Design review of the part built by this model. Coordinates are the model's own, in mm. Face numbers are marked on the shaded views. Round coordinates to 2 decimals unless told otherwise and drop trailing zeros. Loops run counter-clockwise (first coordinate to the right, second up) from the corner with the lowest first, then second, coordinate; pieces in that order, holes last. Notation, with made-up numbers: (52, 16) - (57, 16) arc R29 ccw to (57, 53) - close; hole circle Ø7 at (-29.5, 47). An arc over 180 degrees is marked (long way). Answer as CSV lines item,"result". Start each with the question number.
(1) Consider section C-C (x = 13.5). Give the boundary of the cut face in (y, z).
(2) Consider section A-A (y = 0). Give the boundary of the cut face in (x, z).
(3) Wall thickness on L1, parallel to Y at x = 50, z = 56.4; L2, parallel to Z at x = 0, y = 2.5: over which ranges is each line inside the solid? List them lowest first.
(4) Consider section B-B (z = -28). Give the boundary of the cut face in (x, y), and give its area (3 significant figures).
(5) Mouldability with a two-part tool opening along Z and no side actions: class the marked faces 1 and 2 as released by +Z, released by -Z, zero draft, split by the parting line, or undercut.
(6) For P1, Ø8, axis at y = -7.5, z = -10, coming from the +X side; P2, Ø1.5, axis at y = 1.5, z = 43.5, coming from the +X side; P3, Ø3, axis at x = 50, y = 5.5, coming from the -Z side, all flat-tipped, find the tip position at first contact; note any pin that passes through.
(7) Consider section D-D (x = 50). Give the boundary of the cut face in (y, z), and give its area (3 significant figures).
from build123d import *

# Parameters (mm, degrees)
EXTRUDE_1_DEPTH     = 12.5
SKETCH_3_R          = 2
CUT_EXTRUDE_1_DEPTH = 2


with BuildPart() as part:
    # 草图1 → 拉伸-薄壁1 (new, symmetric)
    with BuildSketch(Plane(origin=(0, 0, 0), x_dir=(1, 0, 0), z_dir=(0, 1, 0))):
        with BuildLine():
            ThreePointArc((23.666622657, -50.753236074), (-12.120618381, 54.672576399), (0, -56))
            Line((0, -56), (60, -56))
            Line((60, -56), (60, -58))
            Line((60, -58), (0, -58))
            ThreePointArc((0, -58), (-12.553497608, 56.625168413), (24.511859181, -52.565851648))
            Line((24.511859181, -52.565851648), (23.666622657, -50.753236074))
        make_face()
    extrude(amount=EXTRUDE_1_DEPTH, both=True)

    # 草图3 → 切除-拉伸1 (cut)
    with BuildSketch(Plane.XY.offset(58)):
        with Locations((50, 5.5)):
            Circle(SKETCH_3_R)
        with Locations(Location((50, -5.5, 0), (0, 0, 180))):
            Circle(SKETCH_3_R)
        with BuildLine():
            Line((15.5, 5.5), (29.5, 5.5))
            ThreePointArc((29.5, 5.5), (35, 0), (29.5, -5.5))
            Line((29.5, -5.5), (15.5, -5.5))
            ThreePointArc((15.5, -5.5), (10, 0), (15.5, 5.5))
        make_face()
    extrude(amount=-CUT_EXTRUDE_1_DEPTH, mode=Mode.SUBTRACT)


solid = part.part
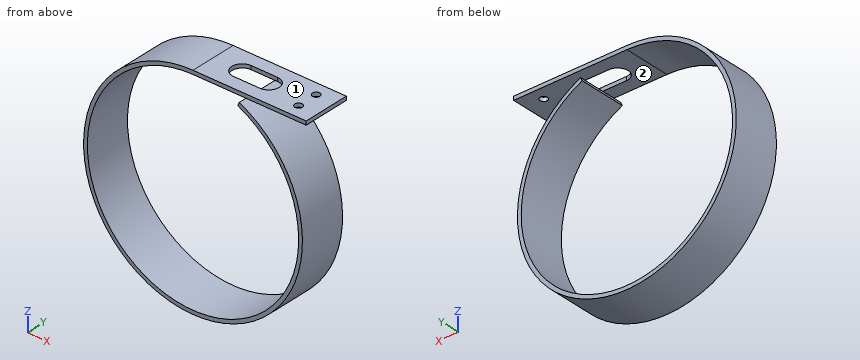
Determined:
1,outline,"(-12.5, -56.41) - (12.5, -56.41) - (12.5, -54.35) - (-12.5, -54.35) - close; (-12.5, 56) - (-5.12, 56) - (-5.12, 58) - (-12.5, 58) - close; (5.12, 56) - (12.5, 56) - (12.5, 58) - (5.12, 58) - close"
2,outline,"(0, 56) - (10, 56) - (10, 58) - (0, 58) arc R58 ccw (long way) to (24.51, 52.57) - (23.67, 50.75) arc R56 cw (long way) to start; (35, 56) - (60, 56) - (60, 58) - (35, 58) - close"
3,L1,"y = -12.5 to -7.5, -3.5 to 3.5, 7.5 to 12.5"
3,L2,"z = -58 to -56, 56 to 58"
4,outline,"(-50.79, -12.5) - (-48.5, -12.5) - (-48.5, 12.5) - (-50.79, 12.5) - close; (48.5, -12.5) - (50.79, -12.5) - (50.79, 12.5) - (48.5, 12.5) - close"
4,area,"115 mm^2"
5,face 1,"released by +Z"
5,face 2,"undercut"
6,P1,"stops at x = 57.69"
6,P2,"stops at x = 39.2"
6,P3,"stops at z = -31.81"
7,outline,"(-12.5, -29.39) - (12.5, -29.39) - (12.5, -25.22) - (-12.5, -25.22) - close; (-12.5, 25.22) - (12.5, 25.22) - (12.5, 29.39) - (-12.5, 29.39) - close; (-12.5, 56) - (-7.5, 56) - (-7.5, 58) - (-12.5, 58) - close; (-3.5, 56) - (3.5, 56) - (3.5, 58) - (-3.5, 58) - close; (7.5, 56) - (12.5, 56) - (12.5, 58) - (7.5, 58) - close"
7,area,"243 mm^2"
